Could you check a few things on this drawing? It's one solid part, dimensions in mm from its lowest x, y, z. A direction names the side the tool comes from. Round coordinates to 2 decimals unless told otherwise and drop trailing zeros. Write each loop counter-clockwise with the first axis right and the second up, starting at its lowest first coordinate (ties: lowest second). Pieces come first, ordered by that corner, then holes. Notation, with made-up numbers: (-24, 1) -> (10, 1) arc R24 ccw to (10, 35) -> close; hole circle Ø6 at (-20, -9). An arc over 180 degrees is marked (long way). Return JSON: item names as keys, results as strings.
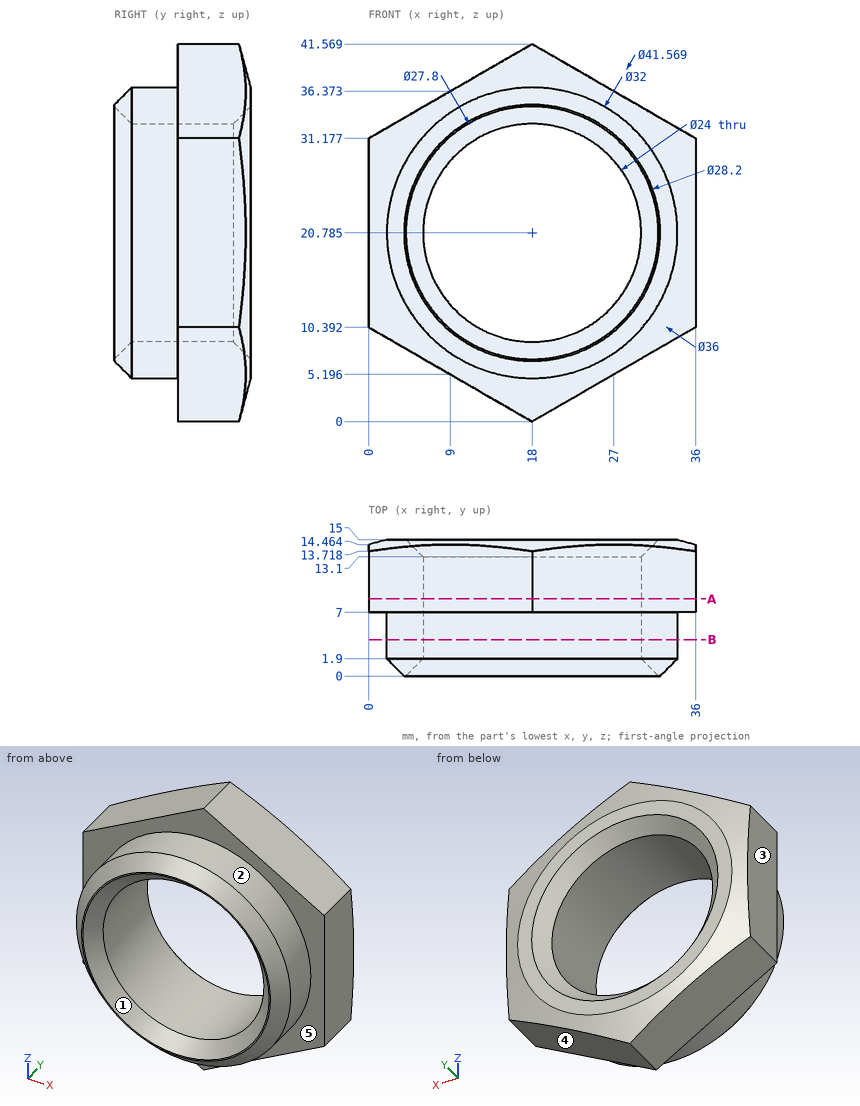
1) I want a section at B-B, the plane y = 4. Please give me the cut outline in (x, z) (1 decimal).
Return value:
{"outline": "circle Ø32 at (18, 20.8); hole circle Ø24 at (18, 20.8)"}
2) For the marked faces 4 and 5, which set-ups out of +Z, -Z, +X, -X, +Y, -Y let a thin tool reach every point of the face, with its end or its side?
Return value:
{"face 4": "-Z, +X, +Y, -Y", "face 5": "-Y"}
3) I want a section at A-A, the plane y = 8.5. Please give me the cut outline in (x, z) (1 decimal).
Return value:
{"outline": "(0, 10.4) -> (18, 0) -> (36, 10.4) -> (36, 31.2) -> (18, 41.6) -> (0, 31.2) -> close; hole circle Ø24 at (18, 20.8)"}
4) If I drill on probe 1 along X at (y, z) = (6, 22); probe 2 along Z at (x, y) = (16.5, 3.25) (1 decimal); probe 3 along Z at (x, y) = (24.5, 10) (1 decimal), over which ranges is the centre line in solid material (lowest first)? Write a range as [from, to].
Return value:
{"probe 1": "[2.05, 6.06], [29.94, 33.95]", "probe 2": "[4.9, 8.9], [32.7, 36.7]", "probe 3": "[3.8, 10.7], [30.9, 37.8]"}
5) Thinking about a two-plate mould opening in X: for the marked faces 1, 2 and 3, which applies, pulls with the +X half, pulls with the -X half, needs draft (parallel to the pull), parting line crosses it, or undercut?
Return value:
{"face 1": "undercut", "face 2": "parting line crosses it", "face 3": "pulls with the -X half"}
6) Will these pins go through, and if not, where does the flat tip stop? pin 1 Ø5 at (y, z) = (3.5, 31.5) entering from -X; pin 2 Ø4 at (x, z) = (10.5, 31.5) entering from -Y; pin 3 Ø19 at (x, z) = (18, 20.78) entering from +Y; pin 4 Ø5 at (x, z) = (14.5, 10) entering from -Y.
Return value:
{"pin 1": "x = 4.27", "pin 2": "y = 0", "pin 3": "through", "pin 4": "y = 0.06"}
